The listing builds one solid part. Answer for the finished solid, in the listing's coordinates (mm). Face numbers are marked on the shaded views. A direction names the side the tool comes from. Round coordinates to 2 decimals unless told otherwise and drop trailing zeros. Order: outer loops, then holes, each group sorted by start corner. A loop starts at its lowest first (then second) coordinate and runs counter-clockwise, first axis right, second up. Notation, with made-up numbers: (32, -4) -> (70, -4) arc R27 cw to (70, 21) -> close; hole circle Ø7 at (86, 31). An arc over 180 degrees is marked (long way). Answer in a Markdown table with one row per item. Add a question column.
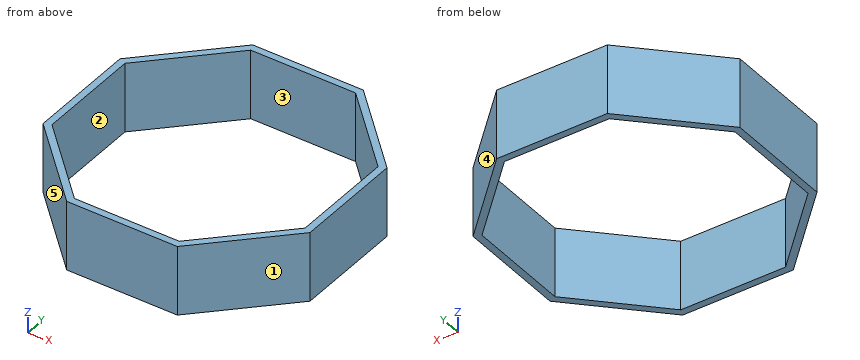
```python
from build123d import *

# Parameters (mm, degrees)
EXTRUDE_1_DEPTH     = 50
CUT_EXTRUDE_1_DEPTH = 606


with BuildPart() as part:
    # 草图1 → 凸台-拉伸1 (new body)
    with BuildSketch(Plane.XY):
        Polygon((-39.799076966, 96.083471381), (-96.083471381, 39.799076966), (-96.083471381, -39.799076966), (-39.799076966, -96.083471381), (39.799076966, -96.083471381), (96.083471381, -39.799076966), (96.083471381, 39.799076966), (39.799076966, 96.083471381), align=None)
    extrude(amount=EXTRUDE_1_DEPTH)

    # 草图2 → 切除-拉伸1 (cut)
    with BuildSketch(Plane.XY.offset(50)):
        Polygon((37.728009154, 91.083471381), (-37.728009154, 91.083471381), (-91.083471381, 37.728009154), (-91.083471381, -37.728009154), (-37.728009154, -91.083471381), (37.728009154, -91.083471381), (91.083471381, -37.728009154), (91.083471381, 37.728009154), align=None)
    extrude(amount=-CUT_EXTRUDE_1_DEPTH, mode=Mode.SUBTRACT)


solid = part.part
```
1. For the marked faces 1 and 2, determine the directions among +Z, -Z, +X, -X, +Y, -Y from which every point of the face is accessible in a straight line to the end or side of a thin tool.
2. Straight lines are drawn through the part: line 1 along Y through (x, z) = (31, 10); line 2 along Y through (x, z) = (-70, 28). For each, find the intervals that lie inside material, in ascending order.
3. The mould has two halves that part along X. Classify the marked faces 3, 4 and 5: released by +X, released by -X, zero draft, split by the parting line, or undercut.
4. The part is cut by section A-A (y = 17.5). Give the vertices of the cut face in (x, z).
5. The part is cut by section C-C (z = 20.5). Give the vertices of the cut face in (x, y).
6. This flat-tipped pin is pushed along its axis until it touches: pin 1 (12 mm diameter, centred on x = -60, z = 10, fed in from +Y). Where does it stop, or does it pass through?
Report:
| question | item | result |
|---|---|---|
| 1 | face 1 | +Z, -Z, +X, -Y |
| 1 | face 2 | +Z, -Z |
| 2 | line 1 | y = -96.08 to -91.08, 91.08 to 96.08 |
| 2 | line 2 | y = -65.88 to -58.81, 58.81 to 65.88 |
| 3 | face 3 | undercut |
| 3 | face 4 | released by +X |
| 3 | face 5 | released by -X |
| 4 | outline | (-96.08, 0) -> (-91.08, 0) -> (-91.08, 50) -> (-96.08, 50) -> close; (91.08, 0) -> (96.08, 0) -> (96.08, 50) -> (91.08, 50) -> close |
| 5 | outline | (-96.08, -39.8) -> (-39.8, -96.08) -> (39.8, -96.08) -> (96.08, -39.8) -> (96.08, 39.8) -> (39.8, 96.08) -> (-39.8, 96.08) -> (-96.08, 39.8) -> close; hole (-91.08, -37.73) -> (-37.73, -91.08) -> (37.73, -91.08) -> (91.08, -37.73) -> (91.08, 37.73) -> (37.73, 91.08) -> (-37.73, 91.08) -> (-91.08, 37.73) -> close |
| 6 | pin 1 | stops at y = 81.88 |
